Job drawing, mm, ordinate dimensions from the low corner. One solid piece. Give positions to 0.01 mm unless a question says otherwise; leave off trailing zeros. Order: outer loops, then holes, each group sorted by start corner. A loop starts at its lowest first (then second) coordinate and runs counter-clockwise, first axis right, second up. Notation, with made-up numbers: (17.25, 22) -> (30.25, 22) arc R27 cw to (30.25, 57) -> close; hole circle Ø2 at (64, -2). An arc over 180 degrees is marked (long way). Write item = value, one per line. Start each with the question number.
(1) Saw through at A-A, the plane y = 15. List the corners of the cut face in (x, z).
(2) Probe line 1 along X through (y, z) = (15, 4.1); line 2 along Y through (x, z) = (15, 4.5); line 3 along X through (y, z) = (14, 1.2). List the from-to ranges inside material, lowest first. Write a range as from..to.
(3) Saw through at C-C, the plane z = 2.15. List the corners of the cut face in (x, y), then the cut area to 3 significant figures.
(4) Flat gauge pin, fed straight in: pin 1 (10 mm diameter, centred on x = 15, y = 15, fed in from -Z). Where does the tip first touch, or does it go through?
(5) Saw through at B-B, the plane x = 55. List the corners of the cut face in (y, z).
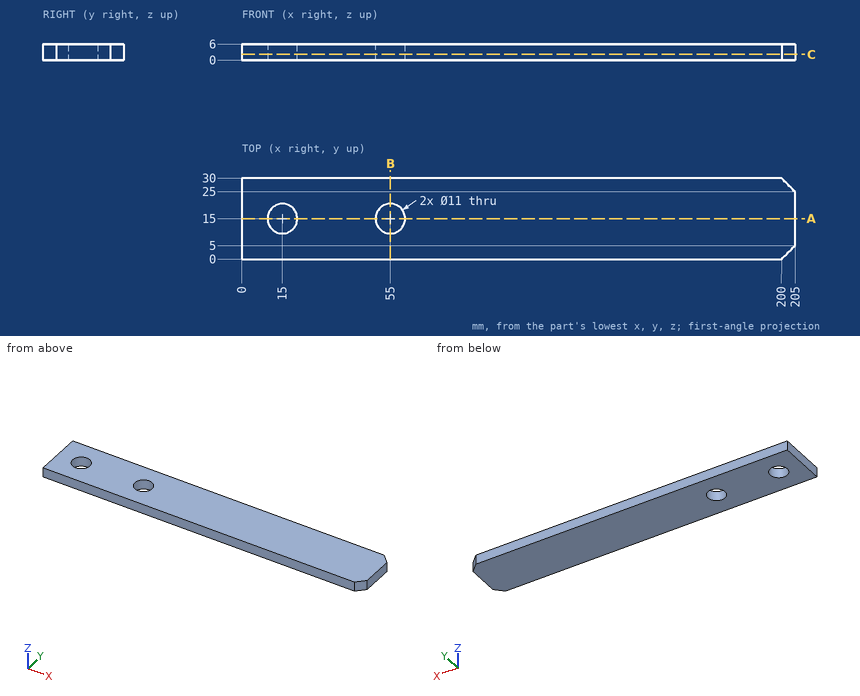
Results list:
q1.outline = (0, 0) -> (9.5, 0) -> (9.5, 6) -> (0, 6) -> close; (20.5, 0) -> (49.5, 0) -> (49.5, 6) -> (20.5, 6) -> close; (60.5, 0) -> (205, 0) -> (205, 6) -> (60.5, 6) -> close
q2.line_1 = 0..9.5, 20.5..49.5, 60.5..205
q2.line_2 = 0..9.5, 20.5..30
q2.line_3 = 0..9.59, 20.41..49.59, 60.41..205
q3.outline = (0, 0) -> (200, 0) -> (205, 5) -> (205, 25) -> (200, 30) -> (0, 30) -> close; hole circle Ø11 at (15, 15); hole circle Ø11 at (55, 15)
q3.area = 5,930 mm^2
q4.pin_1 = through
q5.outline = (0, 0) -> (9.5, 0) -> (9.5, 6) -> (0, 6) -> close; (20.5, 0) -> (30, 0) -> (30, 6) -> (20.5, 6) -> close
